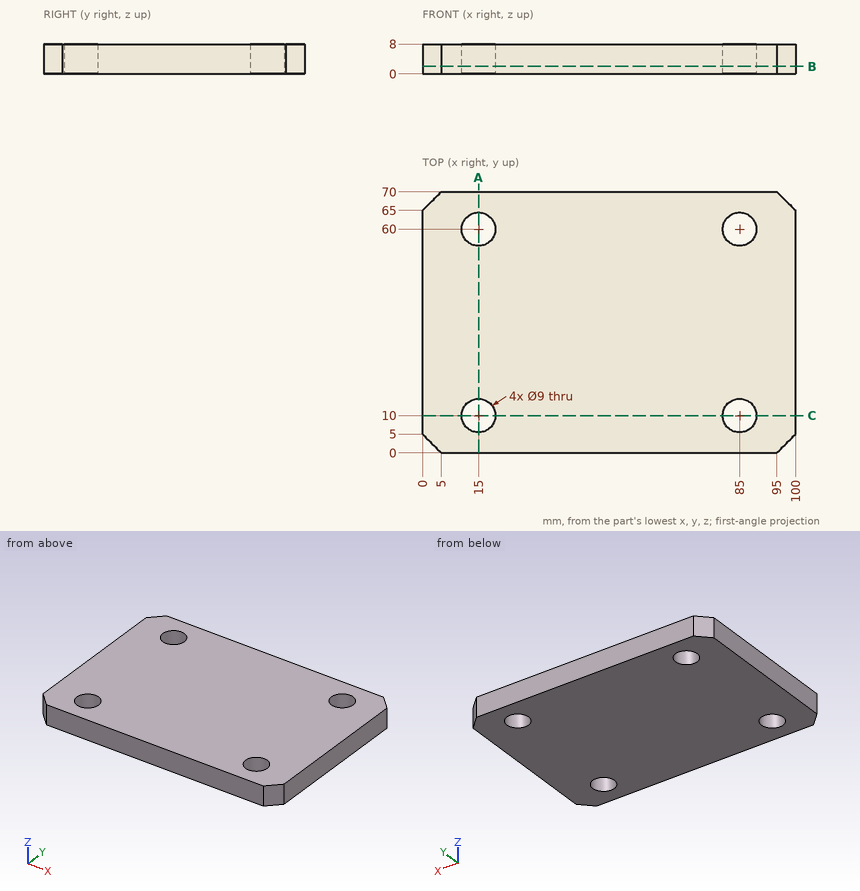
Answer from the drawing. Dimensions are ordinates in mm from the lowest x, y and z of the part. Coordinates: 2 decimals unless noted, no trailing zeros. Loops run counter-clockwise (first coordinate to the right, second up) from the corner with the lowest first, then second, coordinate; pieces in that order, holes last.
Q1. The part is cut by section B-B on z = 2. Write down the section's boundary in (x, y).
Q2. The part is cut by section C-C on y = 10. Write down the section's boundary in (x, z), and give its area (3 significant figures).
Q3. This flat-tipped pin is pushed along its axis until it touches: pin 1 Ø5.5 at (x, y) = (15, 10) entering from -Z. Where does it stop, or does it pass through?
Q4. Consider probe 1 along Y at (x, z) = (85, 2); probe 2 along Y at (x, z) = (82, 7.25). Determine where each line is inside the solid, lowest interval first.
Q5. The part is cut by section A-A on x = 15. Write down the section's boundary in (y, z), and give its area (3 significant figures).
Results below:
1. outline: (0, 5) - (5, 0) - (95, 0) - (100, 5) - (100, 65) - (95, 70) - (5, 70) - (0, 65) - close; hole circle Ø9 at (15, 10); hole circle Ø9 at (15, 60); hole circle Ø9 at (85, 10); hole circle Ø9 at (85, 60)
2. outline: (0, 0) - (10.5, 0) - (10.5, 8) - (0, 8) - close; (19.5, 0) - (80.5, 0) - (80.5, 8) - (19.5, 8) - close; (89.5, 0) - (100, 0) - (100, 8) - (89.5, 8) - close
2. area: 656 mm2
3. pin 1: passes through
4. probe 1: y = 0 to 5.5, 14.5 to 55.5, 64.5 to 70
4. probe 2: y = 0 to 6.65, 13.35 to 56.65, 63.35 to 70
5. outline: (0, 0) - (5.5, 0) - (5.5, 8) - (0, 8) - close; (14.5, 0) - (55.5, 0) - (55.5, 8) - (14.5, 8) - close; (64.5, 0) - (70, 0) - (70, 8) - (64.5, 8) - close
5. area: 416 mm2
